Check sheet for the drawn part. Datum: minimum x, y, z corner. Units: mm. A direction names the side the tool comes from. Give positions to 0.01 mm unless a question says otherwise; leave off trailing zeros. Loops run counter-clockwise (first coordinate to the right, second up) from the corner with the lowest first, then second, coordinate; pieces in that order, holes last. Notation, with made-up numbers: (-6, -24.75) -> (49, -24.75) arc R21 cw to (49, 1.25) -> close; hole circle Ø6 at (68, -7). An arc over 180 degrees is marked (long way). One line per question, with ' | ' between items.
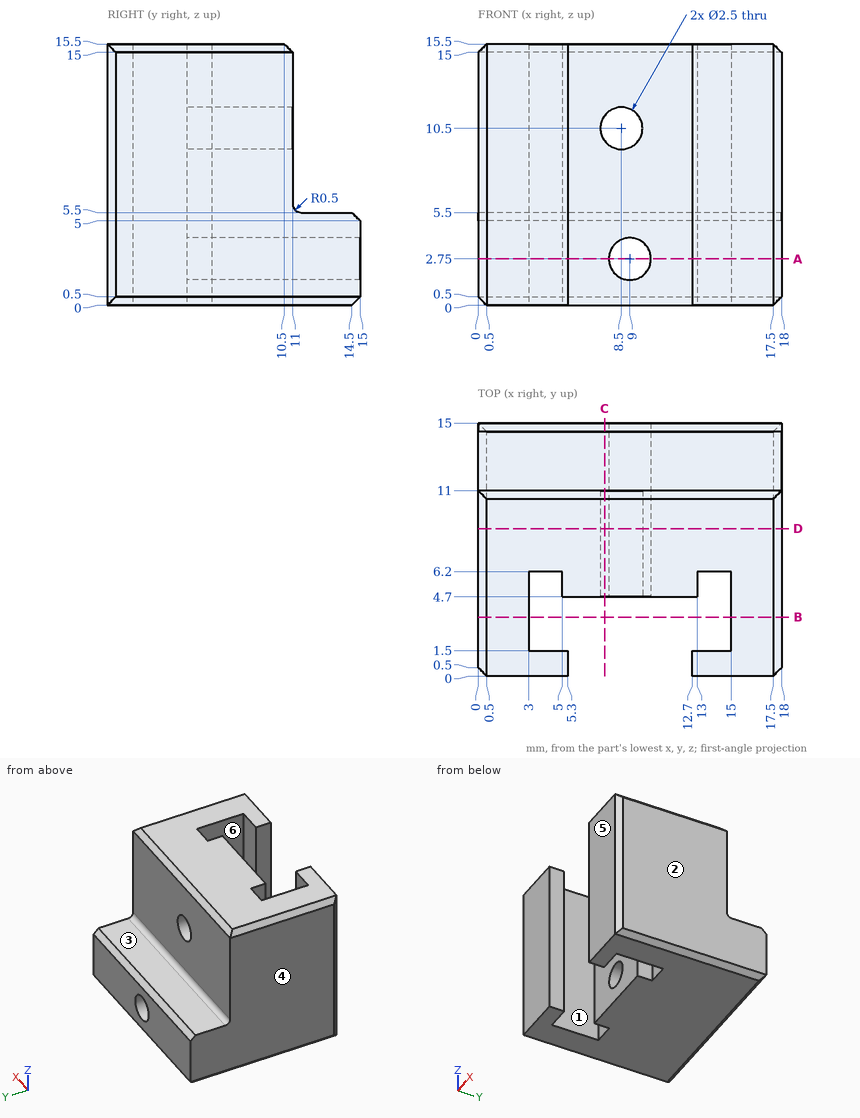
Item 1: Depth check by flat-ended pin: pin 1 Ø2.5 at (x, y) = (11, 12.5) entering from +Z; pin 2 Ø1.2 at (x, z) = (14, 9.5) entering from +Y; pin 3 Ø6 at (y, z) = (13, 10) entering from +X; pin 4 Ø4 at (x, z) = (10.5, 9.5) entering from -Y. Enter the tip coordinate at first touch or a pass-through.
Result:
pin 1: z = 5.57 | pin 2: y = 11 | pin 3: x = 18 | pin 4: y = 4.7
Item 2: Sectioned sample at A-A (z = 2.75). Record the cut outline in (x, y).
Result:
outline: (0, 0.5) -> (0.5, 0) -> (5.3, 0) -> (5.3, 1.5) -> (3, 1.5) -> (3, 6.2) -> (5, 6.2) -> (5, 4.7) -> (7.75, 4.7) -> (7.75, 15) -> (0, 15) -> close; (10.25, 4.7) -> (13, 4.7) -> (13, 6.2) -> (15, 6.2) -> (15, 1.5) -> (12.7, 1.5) -> (12.7, 0) -> (17.5, 0) -> (18, 0.5) -> (18, 15) -> (10.25, 15) -> close
Item 3: Sectioned sample at B-B (y = 3.5). Record the cut outline in (x, z).
Result:
outline: (0, 0.5) -> (0.5, 0) -> (3, 0) -> (3, 15.5) -> (0.5, 15.5) -> (0, 15) -> close; (15, 0) -> (17.5, 0) -> (18, 0.5) -> (18, 15) -> (17.5, 15.5) -> (15, 15.5) -> close
Item 4: Scan lines: probe 1 along X at (y, z) = (4.75, 5.5); probe 2 along Y at (x, z) = (4.75, 13); probe 3 along X at (y, z) = (12, 2.75). Record each from-to range of solid material in increasing order.
Result:
probe 1: 0 to 3, 5 to 13, 15 to 18 | probe 2: 0 to 1.5, 6.2 to 11 | probe 3: 0 to 7.75, 10.25 to 18
Item 5: Sectioned sample at C-C (x = 7.5). Record the cut outline in (y, z).
Result:
outline: (4.7, 0) -> (14.5, 0) -> (15, 0.5) -> (15, 5) -> (14.5, 5.5) -> (11.5, 5.5) arc R0.5 cw to (11, 6) -> (11, 9.75) -> (4.7, 9.75) -> close; (4.7, 11.25) -> (11, 11.25) -> (11, 15) -> (10.5, 15.5) -> (4.7, 15.5) -> close
Item 6: Release check for a two-part mould opening along X. For the marked faces 4, 5 and 6 record: pulls with the +X half, pulls with the -X half, needs draft (parallel to the pull), parting line crosses it, or undercut.
Result:
face 4: pulls with the -X half | face 5: needs draft | face 6: undercut
Item 7: Set-up check for the marked faces 1, 2 and 3: record each of +Z, -Z, +X, -X, +Y, -Y from which the full face is reachable in a straight line by a thin tool's end or side.
Result:
face 1: +Z, -Z | face 2: +Z, -Z, +X, +Y, -Y | face 3: +Z, +X, -X, +Y
Item 8: Sectioned sample at D-D (y = 8.75). Record the cut outline in (x, z), plus the area to 3 significant figures.
Result:
outline: (0, 0.5) -> (0.5, 0) -> (17.5, 0) -> (18, 0.5) -> (18, 15) -> (17.5, 15.5) -> (0.5, 15.5) -> (0, 15) -> close; hole circle Ø2.5 at (8.5, 10.5); hole circle Ø2.5 at (9, 2.75) | area: 269 mm2
